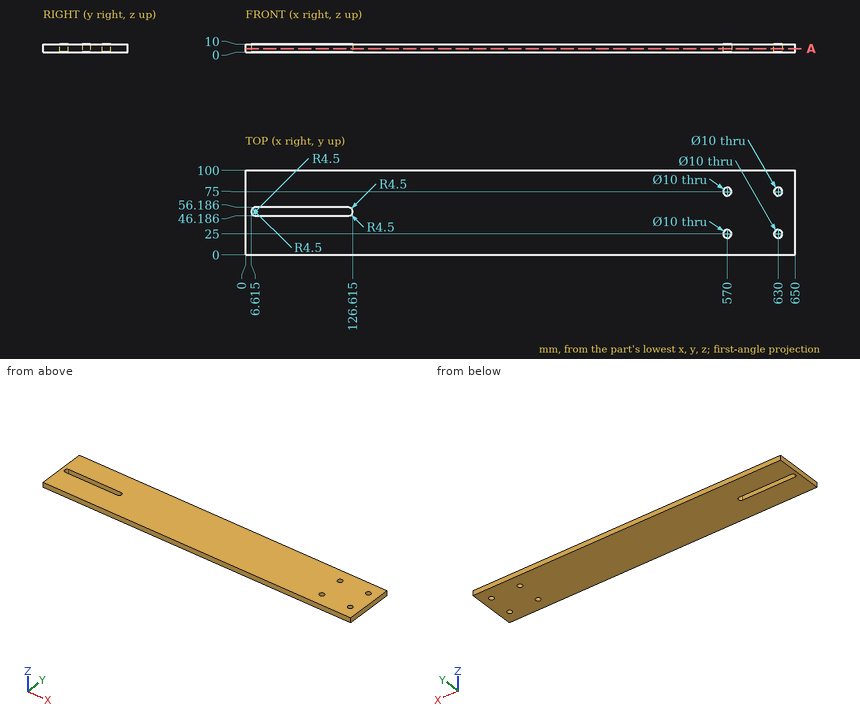
Answer from the drawing. Dimensions are ordinates in mm from the lowest x, y and z of the part. Round coordinates to 2 decimals unless told otherwise and drop trailing zeros. Write each loop counter-clockwise with the first axis right and the second up, starting at its lowest first coordinate (ties: lowest second). Pieces come first, ordered by that corner, then holes. Notation, with made-up numbers: (-31, 20) - (8, 20) arc R19 ccw to (8, 50) - close; hole circle Ø10 at (1, -5). An arc over 180 degrees is marked (long way). Use a Markdown table: item, result.
(1) Straight lines are drawn through the part: line 1 along Y through (x, z) = (630, 7.75); line 2 along Y through (x, z) = (118.5, 3.25) (1 decimal); line 3 along X through (y, z) = (53.5, 8). For each, find the intervals that lie inside material, in ascending order. Write a range as [from, to].
Reported:
| item | result |
|---|---|
| line 1 | [0, 20], [30, 70], [80, 100] |
| line 2 | [0, 46.2], [56.2, 100] |
| line 3 | [0, 7], [126.23, 650] |
(2) The part is cut by section A-A (z = 4.5). Write down the section's boundary in (x, y) (1 decimal).
Reported:
| item | result |
|---|---|
| outline | (0, 0) - (650, 0) - (650, 100) - (0, 100) - close; hole (6.6, 50.7) arc R4.5 ccw to (11.1, 46.2) - (122.1, 46.2) arc R4.5 ccw to (126.6, 50.7) - (126.6, 51.7) arc R4.5 ccw to (122.1, 56.2) - (11.1, 56.2) arc R4.5 ccw to (6.6, 51.7) - close; hole circle Ø10 at (570, 25); hole circle Ø10 at (570, 75); hole circle Ø10 at (630, 25); hole circle Ø10 at (630, 75) |
(3) This flat-tipped pin is pushed along its axis until it touches: pin 1 Ø5 at (x, z) = (68, 7.5) entering from -Y. Where does it stop, or does it pass through?
Reported:
| item | result |
|---|---|
| pin 1 | y = 0 |
